The figure shows three views and two pictorial views of one solid part (mm, origin at its lowest corner). Answer the questions. A direction names the side the tool comes from. Coordinates: 2 decimals unless noted, no trailing zeros. Order: outer loops, then holes, each group sorted by start corner. A loop starts at its lowest first (then second) coordinate and runs counter-clockwise, first axis right, second up. Notation, with made-up numbers: (44.25, 41.25) -> (57.25, 41.25) arc R17 cw to (57.25, 55.25) -> close; hole circle Ø7 at (-2, 18.25). An arc over 180 degrees is marked (long way). Write item = value, one per line.
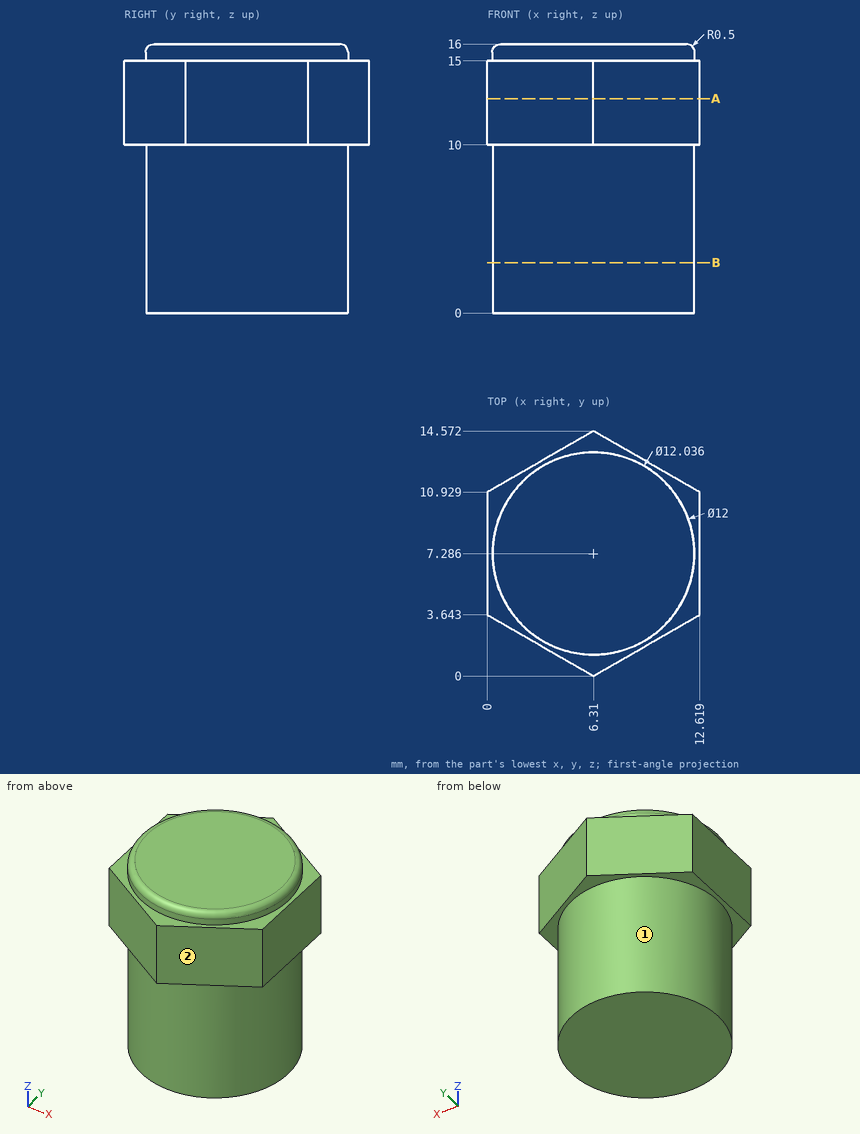
Q1. Section B-B, the plane z = 3 is taken. Give the vertices of the cut face in (x, y) (1 decimal).
The answers:
outline = circle Ø12 at (6.3, 7.3)
Q2. A tool of negligible diameter and unlimited length cuts with its end or side. For the marked faces 1 and 2, from which of +Z, -Z, +X, -X, +Y, -Y can it reach the whole face along a straight path? Write none if from no direction.
The answers:
face_1 = -Z
face_2 = +Z, -Z, +X, -Y
Q3. Section A-A, the plane z = 12.75 is taken. Give the vertices of the cut face in (x, y).
The answers:
outline = (0, 3.64) -> (6.31, 0) -> (12.62, 3.64) -> (12.62, 10.93) -> (6.31, 14.57) -> (0, 10.93) -> close
Q4. Find the intervals of material crossed by line 1 along Z through (x, y) = (10.25, 12); line 2 along X through (y, z) = (2.5, 6.75); line 3 along X through (y, z) = (9, 1.25), in increasing order.
The answers:
line_1 = 10 to 15
line_2 = 2.69 to 9.93
line_3 = 0.56 to 12.06
Q5. Each of these flat-tipped pins is pushed along its axis until it touches: pin 1 Ø1.5 at (x, z) = (10.5, 7) entering from -Y; pin 2 Ø4 at (x, z) = (5, 1.5) entering from +Y; pin 3 Ø2 at (x, z) = (7.5, 11.5) entering from -Y. Where does it stop, or does it pass through?
The answers:
pin_1 = 2.37
pin_2 = 13.29
pin_3 = 0.11
